Could you check a few things on this model? Use its own coordinates, in mm. A direction names the side the tool comes from. Give positions to 0.01 mm unless a question says otherwise; leave off trailing zeros. Write each loop counter-clockwise with the first axis right and the second up, starting at its lowest first coordinate (ties: lowest second). Pieces come first, ordered by that corner, then holes. Notation, with made-up numbers: (6.5, 62) - (35.5, 62) arc R32 ccw to (35.5, 99) - close; hole circle Ø1 at (-30, -21). An arc over 180 degrees is marked (long way). Write item = value, one per line.
from build123d import *

# Parameters (mm, degrees)
BOSS_EXTRUDE1_DEPTH = 400


with BuildPart() as part:
    # Sketch1 → Boss-Extrude1 (new body)
    with BuildSketch(Plane.XY):
        with BuildLine():
            Line((0, 70), (0, 0))
            Line((0, 0), (70, 0))
            Line((70, 0), (70, 5))
            ThreePointArc((70, 5), (69.121320344, 7.121320344), (67, 8))
            Line((67, 8), (16, 8))
            ThreePointArc((16, 8), (10.343145751, 10.343145751), (8, 16))
            Line((8, 16), (8, 67))
            ThreePointArc((8, 67), (7.121320344, 69.121320344), (5, 70))
            Line((5, 70), (0, 70))
        make_face()
    extrude(amount=BOSS_EXTRUDE1_DEPTH)


solid = part.part
1. Which directions (+Z, -Z, +X, -X, +Y, -Y) give clear straight access to the entire face, cutting with the end or side of a thin tool? Please do faces 1 (the face through (42, 8, 197)), 2 (the face through (6, 22, 400)).
Filled sheet:
face_1 = +Z, -Z, +X, +Y
face_2 = +Z, +X, -X, +Y, -Y
2. If we section it at A-A, the plane z = 185: Please give me the cut outline in (x, y), and give its area (3 significant figures).
Filled sheet:
outline = (0, 0) - (70, 0) - (70, 5) arc R3 ccw to (67, 8) - (16, 8) arc R8 cw to (8, 16) - (8, 67) arc R3 ccw to (5, 70) - (0, 70) - close
area = 1,070 mm2
3. I need wall thicknesses on line 1 (Y direction, x = 22.5, z = 349.5); line 2 (Y direction, x = 13.5, z = 362.5). Which ranges of each line are inside material? Lowest first, please.
Filled sheet:
line_1 = 0 to 8
line_2 = 0 to 8.4
4. For pin 1 (6 mm diameter, centred on x = 41, z = 53.5, fed in from +Y); pin 2 (5 mm diameter, centred on y = 59.5, z = 58.5, fed in from +X); pin 3 (1 mm diameter, centred on y = 35.5, z = 133, fed in from -X); pin 4 (1 mm diameter, centred on x = 7.5, z = 46, fed in from +Y), each with a flat end and sliding along its axis, tell me the tip position at first contact or that it passes through.
Filled sheet:
pin_1 = 8
pin_2 = 8
pin_3 = 0
pin_4 = 69.24
5. If we section it at B-B, the plane y = 28: Please give me the cut outline in (x, z).
Filled sheet:
outline = (0, 0) - (8, 0) - (8, 400) - (0, 400) - close
